from build123d import *

# Parameters (mm, degrees)
SKETCH_1_W                = 60
SKETCH_1_H                = 50
EXTRUDE_1_DEPTH           = 10
SKETCH_5_W                = 31
SKETCH_5_H                = 50
CUT_EXTRUDE_1_DEPTH       = 1
CHAMFER_2_SIZE            = 3
HOLE_WIZARD_M5_1_D        = 4.2
HOLE_WIZARD_M5_1_DEPTH    = 12.4
HOLE_WIZARD_M5_1_TIP      = 1.2618073
HOLE_WIZARD_3_D           = 3.4
HOLE_WIZARD_3_DEPTH       = 12.4
HOLE_WIZARD_3_CBORE_D     = 6
HOLE_WIZARD_3_CBORE_DEPTH = 3.4
HOLE_WIZARD_3_TIP         = 1.021463052
MM_3_D                    = 4
MM_3_DEPTH                = 12.4
MM_3_TIP                  = 1.201721238


with BuildPart() as part:
    # 草图1 → 凸台-拉伸1 (new body)
    with BuildSketch(Plane(origin=(0, 0, 0), x_dir=(1, 0, 0), z_dir=(0, 1, 0))):
        Rectangle(SKETCH_1_W, SKETCH_1_H)
    extrude(amount=EXTRUDE_1_DEPTH)

    # 草图5 → 切除-拉伸1 (cut)
    with BuildSketch(Plane.XZ):
        with Locations((14.5, 0)):
            Rectangle(SKETCH_5_W, SKETCH_5_H)
    extrude(amount=-CUT_EXTRUDE_1_DEPTH, mode=Mode.SUBTRACT)

    # 倒角2
    chamfer_2_edges = [part.edges().sort_by_distance(p)[0] for p in [
        (30, 5.5, 25),
        (-30, 5, 25),
        (-30, 5, -25),
        (30, 5.5, -25),
    ]]
    chamfer(chamfer_2_edges, length=CHAMFER_2_SIZE)

    # M5 螺纹孔1
    with Locations(Plane.ZY.offset(30)):
        with Locations((17, 5), (-17, 4.974257895), (0, 4.974257895)):
            Hole(HOLE_WIZARD_M5_1_D / 2, depth=HOLE_WIZARD_M5_1_DEPTH)
            with Locations((0, 0, -(HOLE_WIZARD_M5_1_DEPTH + HOLE_WIZARD_M5_1_TIP / 2))):  # 118° drill point
                Cone(0, HOLE_WIZARD_M5_1_D / 2, HOLE_WIZARD_M5_1_TIP, mode=Mode.SUBTRACT)

    # 打孔尺寸(%根据)内六角圆柱头螺钉的类型3
    with Locations(Plane(origin=(0, 10, 0), x_dir=(1, 0, 0), z_dir=(0, 1, 0))):
        with Locations((23.5, -18), (3.5, -18), (13.5, 5.7)):
            CounterBoreHole(HOLE_WIZARD_3_D / 2, HOLE_WIZARD_3_CBORE_D / 2, HOLE_WIZARD_3_CBORE_DEPTH, depth=HOLE_WIZARD_3_DEPTH)
            with Locations((0, 0, -(HOLE_WIZARD_3_DEPTH + HOLE_WIZARD_3_TIP / 2))):  # 118° drill point
                Cone(0, HOLE_WIZARD_3_D / 2, HOLE_WIZARD_3_TIP, mode=Mode.SUBTRACT)

    # 大小mm 暗销孔3
    with Locations(Plane.ZY.offset(30)):
        with Locations((9, 5), (-9, 5)):
            Hole(MM_3_D / 2, depth=MM_3_DEPTH)
            with Locations((0, 0, -(MM_3_DEPTH + MM_3_TIP / 2))):  # 118° drill point
                Cone(0, MM_3_D / 2, MM_3_TIP, mode=Mode.SUBTRACT)


solid = part.part
Check sheet for the modelled part. Datum: model origin and axes. Units: mm. A direction names the side the tool comes from. Give positions to 0.01 mm unless a question says otherwise; leave off trailing zeros. Loops run counter-clockwise (first coordinate to the right, second up) from the corner with the lowest first, then second, coordinate; pieces in that order, holes last. Notation, with made-up numbers: M 21.5,52.5 L 74.5,52.5 A27 cw 74.5,90.5 Z; hole C 61.5,12.5 d10. An arc over 180 degrees is marked long. Return JSON: item names as keys, results as strings. Group by question number.
1. Cross-section at D-D on z = 13. Record the boundary of the cut face in (x, y).
2. Cross-section at B-B on x = 13.5. Record the boundary of the cut face in (y, z).
3. Go/stop test with flat-tipped pins: pin 1 (4 mm diameter, centred on x = 3.5, z = 18, fed in from +Y); pin 2 (3 mm diameter, centred on y = 5, z = 9, fed in from -X); pin 3 (5.5 mm diameter, centred on x = 13.5, z = -5.7, fed in from -Y). Record where each tip stops, or that it passes through.
4. Mould release check, pull along Z, two halves, no side actions. Record for faces 4 (the cylindrical face through (-23.713, 5.631, 14.997)), 5 (the flat face through (-16, 0, 0)), 6 (the flat face through (29, 5, -23)): released by +Z, released by -Z, zero draft, split by the parting line, or undercut.
5. Tool access check on faces 1 (the cylindrical face through (2.85, 8.32, 20.93)), 2 (the flat face through (30, 5, 0)), 3 (the cylindrical face through (-24, 5, -7)). Record the directions out of +Z, -Z, +X, -X, +Y, -Y that give a thin tool (end or side, any length) a straight path to the whole face; none if there is none.
6. Cross-section at A-A on z = -5.7. Record the boundary of the cut face in (x, y).
7. Thickness scan on L1, parallel to Z at x = -18.5, y = 4.75; L2, parallel to X at y = 8.8, z = 18; L3, parallel to Y at x = -22.25, z = 9. Record the ranges inside material, lowest first.
8. Cross-section at C-C on y = 8.75. Record the boundary of the cut face in (x, z).
Return value:
{
 "1": {"outline": "M -30,0 L -1,0 L -1,1 L 30,1 L 30,10 L -30,10 Z"},
 "2": {"outline": "M 1,-25 L 10,-25 L 10,-8.7 L 6.6,-8.7 L 6.6,-7.4 L 1,-7.4 Z; M 1,-4 L 6.6,-4 L 6.6,-2.7 L 10,-2.7 L 10,25 L 1,25 Z"},
 "3": {"pin 1": "y = 6.6", "pin 2": "x = -17.3", "pin 3": "y = 1"},
 "4": {"face 4": "undercut", "face 5": "zero draft", "face 6": "released by -Z"},
 "5": {"face 1": "+Y", "face 2": "+Z, -Z, +X, +Y, -Y", "face 3": "-X"},
 "6": {"outline": "M -30,0 L -1,0 L -1,1 L 11.8,1 L 11.8,6.6 L 10.5,6.6 L 10.5,10 L -30,10 Z; M 15.2,1 L 30,1 L 30,10 L 16.5,10 L 16.5,6.6 L 15.2,6.6 Z"},
 "7": {"L1": "-25 to -19.09, -14.91 to -10.98, -7.02 to -2.09, 2.09 to 7.02, 10.98 to 14.91, 19.09 to 25", "L2": "-30 to 0.5, 6.5 to 20.5, 26.5 to 30", "L3": "0 to 3, 7 to 10"},
 "8": {"outline": "M -30,-22 L -27,-25 L 27,-25 L 30,-22 L 30,22 L 27,25 L -27,25 L -30,22 Z; hole C 3.5,18 d6; hole C 13.5,-5.7 d6; hole C 23.5,18 d6"}
}
